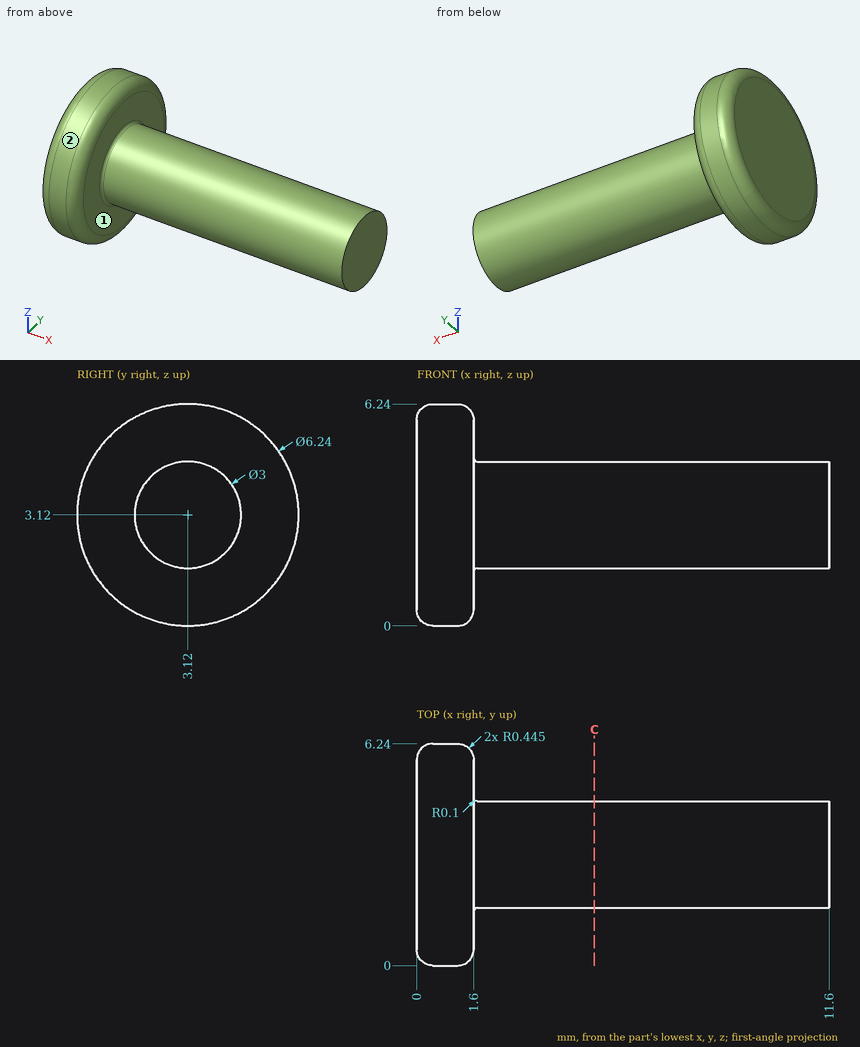
Could you check a few things on this drawing? It's one solid part, dimensions in mm from its lowest x, y, z. A direction names the side the tool comes from. Round coordinates to 2 decimals unless told otherwise and drop trailing zeros. Order: outer loops, then holes, each group sorted by start corner. A loop starts at its lowest first (then second) coordinate and runs counter-clockwise, first axis right, second up.
(1) I'm going to push flat-ended pins straight in: pin 1 (3 mm diameter, centred on y = 1, z = 1, fed in from -X); pin 2 (1.5 mm diameter, centred on x = 5, z = 2, fed in from -Y). Where does each tip first touch, or does it pass through?
Response values:
pin 1: stops at x = 0
pin 2: stops at y = 1.67
(2) Imagine slicing it at C-C (x = 5). Write out the boundary of the cut face in (y, z).
Response values:
outline: circle Ø3 at (3.12, 3.12)
(3) Please list where these lines run through material, in increasing order: line 1 along X through (y, z) = (1.5, 3.75); line 2 along Z through (x, y) = (8.5, 2.5); line 3 along Y through (x, z) = (4.75, 1.75).
Response values:
line 1: x = 0 to 1.6
line 2: z = 1.75 to 4.49
line 3: y = 2.51 to 3.73
(4) Which directions (+Z, -Z, +X, -X, +Y, -Y) give clear straight access to the entire face, cutting with the end or side of a thin tool? Please do the marked faces 1 and 2.
Response values:
face 1: +X
face 2: +X, -X
